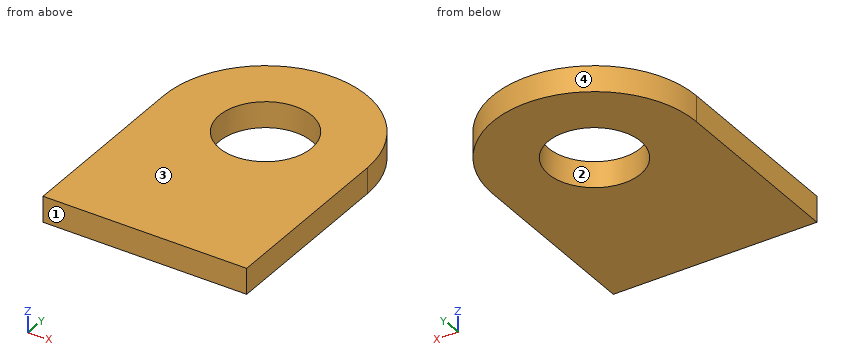
```python
from build123d import *

# Parameters (mm, degrees)
SKETCH1_R           = 25
BOSS_EXTRUDE1_DEPTH = 14


with BuildPart() as part:
    # Sketch1 → Boss-Extrude1 (new body)
    with BuildSketch(Plane.XY):
        with BuildLine():
            Line((-55, 0), (-55, -100))
            Line((-55, -100), (55, -100))
            Line((55, -100), (55, 0))
            ThreePointArc((55, 0), (0, 55), (-55, 0))
        make_face()
        Circle(SKETCH1_R, mode=Mode.SUBTRACT)
    extrude(amount=BOSS_EXTRUDE1_DEPTH)


solid = part.part
```
For this review, take the finished solid that the model builds, in its own axes (mm). Face numbers are marked on the shaded views. Round coordinates to 2 decimals unless told otherwise and drop trailing zeros. Write each loop counter-clockwise with the first axis right and the second up, starting at its lowest first coordinate (ties: lowest second). Pieces come first, ordered by that corner, then holes. Notation, with made-up numbers: (29.5, 30) - (76.5, 30) arc R24 cw to (76.5, 67) - close; hole circle Ø10 at (-26.5, 80.25). An arc over 180 degrees is marked (long way). Answer as CSV lines item,"result". Start each with the question number.
(1) For pin 1 (1 mm diameter, centred on x = -19.5, z = 5, fed in from +Y), flat-tipped, find the tip position at first contact; note if it passes through.
(2) Add section B-B, the plane y = -13. State the section outline as (x, z) points.
(3) Add section C-C, the plane z = 11.75. State the section outline as (x, y) points, plus the area to 3 significant figures.
(4) Add section D-D, the plane x = -37.5. State the section outline as (y, z) points.
(5) Mouldability with a two-part tool opening along Y and no side actions: class the marked faces 1, 2, 3 and 4 as +Y half, -Y half, draft (parallel to the pull), parting line (faces both ways), or undercut.
(6) Add section A-A, the plane x = 0. State the section outline as (y, z) points, plus the area to 3 significant figures.
(7) For line 1 (Y direction, x = 1, z = 10); line 2 (Y direction, x = -10.5, z = 10.25); line 3 (X direction, y = 26.5, z = 10), list the stretches that pass through material, from the lowest coordinate up.
From the geometry:
1,pin 1,"stops at y = 51.61"
2,outline,"(-55, 0) - (-21.35, 0) - (-21.35, 14) - (-55, 14) - close; (21.35, 0) - (55, 0) - (55, 14) - (21.35, 14) - close"
3,outline,"(-55, -100) - (55, -100) - (55, 0) arc R55 ccw to (-55, 0) - close; hole circle Ø50 at (0, 0)"
3,area,"13,800 mm²"
4,outline,"(-100, 0) - (40.23, 0) - (40.23, 14) - (-100, 14) - close"
5,face 1,"-Y half"
5,face 2,"undercut"
5,face 3,"draft"
5,face 4,"+Y half"
6,outline,"(-100, 0) - (-25, 0) - (-25, 14) - (-100, 14) - close; (25, 0) - (55, 0) - (55, 14) - (25, 14) - close"
6,area,"1,470 mm²"
7,line 1,"y = -100 to -24.98, 24.98 to 54.99"
7,line 2,"y = -100 to -22.69, 22.69 to 53.99"
7,line 3,"x = -48.19 to 48.19"
